Read the model definition and answer for the solid it produces. Units are mm, in the model's axes. A direction names the side the tool comes from. Give positions to 0.01 mm unless a question says otherwise; leave off trailing zeros. Order: outer loops, then holes, each group sorted by start corner. A loop starts at its lowest first (then second) coordinate and runs counter-clockwise, first axis right, second up. Notation, with made-up numbers: (28.25, 78) -> (70.25, 78) arc R27 ccw to (70.25, 100) -> close; hole circle Ø6 at (-36, -8). An arc over 180 degrees is marked (long way). One line per item, written item: value. Start each with the question number.
from build123d import *

# Parameters (mm, degrees)
EXTRUDE_1_DEPTH              = 50
HOLE_WIZARD_M8_1_D           = 10
HOLE_WIZARD_M8_1_CSINK_D     = 17.92
HOLE_WIZARD_M8_1_CSINK_ANGLE = 90
MOVE_FACE_1_BY               = 130
HOLE_WIZARD_M8_1_2_D         = 10


with BuildPart() as part:
    # 草图1 → 凸台-拉伸1 (new, symmetric)
    with BuildSketch(Plane.XY):
        Polygon((0, 0), (75, 0), (75, 75), (65, 75), (65, 10), (0, 10), align=None)
    extrude(amount=EXTRUDE_1_DEPTH, both=True)

    # Hole Wizard M8 _1 (through all)
    with Locations(Plane.ZY.offset(-65)):
        with Locations((-40, 65), (35, 65), (-40, 30), (35, 30)):
            CounterSinkHole(HOLE_WIZARD_M8_1_D / 2, HOLE_WIZARD_M8_1_CSINK_D / 2, counter_sink_angle=HOLE_WIZARD_M8_1_CSINK_ANGLE)

    # Move Face 1: a face moved outward by 130.0
    extrude(part.faces().sort_by_distance((37.5, 7.5, -50))[0], amount=MOVE_FACE_1_BY, dir=(0, 0, -1))

    # Hole Wizard M8 _1 2 (through all)
    with Locations(Plane(origin=(0, 10, 0), x_dir=(1, 0, 0), z_dir=(0, 1, 0))):
        with Locations((10.5, 165), (10.5, 95), (44.5, 165), (44.5, 95)):
            Hole(HOLE_WIZARD_M8_1_2_D / 2)


solid = part.part
Item 1: Find section B-B on x = 44.5. Write down the section's boundary in (y, z), then the cut area to 3 significant figures.
Item 2: Find section A-A on z = -165. Write down the section's boundary in (x, y), then the cut area to 3 significant figures.
Item 3: For a pull along X with two mould halves and no side action, classify faces 3 (the flat face through (0, 5, -63)), 4 (the cylindrical face through (72, 68, 39)), 5 (the cylindrical face through (48.5, 4.9, -92)) as +X half, -X half, draft (parallel to the pull), parting line (faces both ways), or undercut.
Item 4: Find the intervals of material crossed by line 1 (Z direction, x = 70.5, y = 65); line 2 (X direction, y = 2, z = -95); line 3 (Y direction, x = 51.5, z = -64.5), in increasing order. Write a range as from..to.
Item 5: Find section D-D on z = 35. Write down the section's boundary in (x, y), then the cut area to 3 significant figures.
Item 6: Find section C-C on y = 30. Write down the section's boundary in (x, z).
Item 7: A tool of negligible diameter and unlimited length cuts with its end or side. For faces 1 (the flat face through (33, 10, -63)), 2 (the cylindrical face through (72, 68, -36)), from which of +Z, -Z, +X, -X, +Y, -Y can it reach the whole face along a straight path? Write none if from no direction.
Item 8: Flat-ended cylindrical pins translate along their axes: pin 1 (8 mm diameter, centred on y = 30, z = 35, fed in from -X); pin 2 (11.5 mm diameter, centred on y = 65, z = -40, fed in from -X); pin 3 (6 mm diameter, centred on y = 42.5, z = -3.5, fed in from -X). Find the tip coordinate at first contact, or state that the pin passes through.
Checks:
1. outline: (0, -180) -> (10, -180) -> (10, -170) -> (0, -170) -> close; (0, -160) -> (10, -160) -> (10, -100) -> (0, -100) -> close; (0, -90) -> (10, -90) -> (10, 50) -> (0, 50) -> close
1. area: 2,100 mm2
2. outline: (0, 0) -> (5.5, 0) -> (5.5, 10) -> (0, 10) -> close; (15.5, 0) -> (39.5, 0) -> (39.5, 10) -> (15.5, 10) -> close; (49.5, 0) -> (75, 0) -> (75, 75) -> (65, 75) -> (65, 10) -> (49.5, 10) -> close
2. area: 1,200 mm2
3. face 3: -X half
3. face 4: draft
3. face 5: undercut
4. line 1: -180..-45, -35..30, 40..50
4. line 2: 0..5.5, 15.5..39.5, 49.5..75
4. line 3: 0..10
5. outline: (0, 0) -> (75, 0) -> (75, 25) -> (68.96, 25) -> (65, 21.04) -> (65, 10) -> (0, 10) -> close; (65, 38.96) -> (68.96, 35) -> (75, 35) -> (75, 60) -> (68.96, 60) -> (65, 56.04) -> close; (65, 73.96) -> (68.96, 70) -> (75, 70) -> (75, 75) -> (65, 75) -> close
5. area: 1,170 mm2
6. outline: (65, -180) -> (75, -180) -> (75, -45) -> (68.96, -45) -> (65, -48.96) -> close; (65, -31.04) -> (68.96, -35) -> (75, -35) -> (75, 30) -> (68.96, 30) -> (65, 26.04) -> close; (65, 43.96) -> (68.96, 40) -> (75, 40) -> (75, 50) -> (65, 50) -> close
7. face 1: +Z, -Z, -X, +Y
7. face 2: +X, -X
8. pin 1: through
8. pin 2: x = 68.21
8. pin 3: x = 65
